Part print with two shaded views. Sizes in mm from the minimum x, y, z corner. Round coordinates to 2 decimals unless told otherwise and drop trailing zeros. Write each loop counter-clockwise with the first axis right and the second up, starting at its lowest first coordinate (ties: lowest second). Pieces come first, ordered by that corner, then holes. Notation, with made-up numbers: M 72,71.25 L 87,71.25 A21 ccw 87,105.25 Z; hole C 33.5,-6 d5. An arc over 180 degrees is marked long. One line per question, with ' | ' between items. Start each with the question number.
1) Saw through at C-C (z = 8.75). List the corners of the cut face in (x, y), plus the area to 3 significant figures.
2) Wall check: probe 1 along X at (y, z) = (135, 9.5); probe 2 along X at (y, z) = (136.5, 7.75); probe 3 along Y at (x, z) = (4.25, 7.25). Give the ranges that are in metal, low to high. Write a range as [from, to].
3) Saw through at B-B (y = 135). List the corners of the cut face in (x, z), plus the area to 4 significant figures.
4) Drop a flat-ended pin along its axis: pin 1 Ø4 at (x, y) = (5.5, 106) entering from -Z. Give the stop position or say it passes through.
5) Mould opens along Y. For the marked faces 1, 2 and 3 say: pulls with the +Y half, pulls with the -Y half, needs draft (parallel to the pull), parting line crosses it, or undercut.
6) Saw through at A-A (x = 15). List the corners of the cut face in (y, z).
7) Saw through at D-D (y = 28.5). List the corners of the cut face in (x, z).
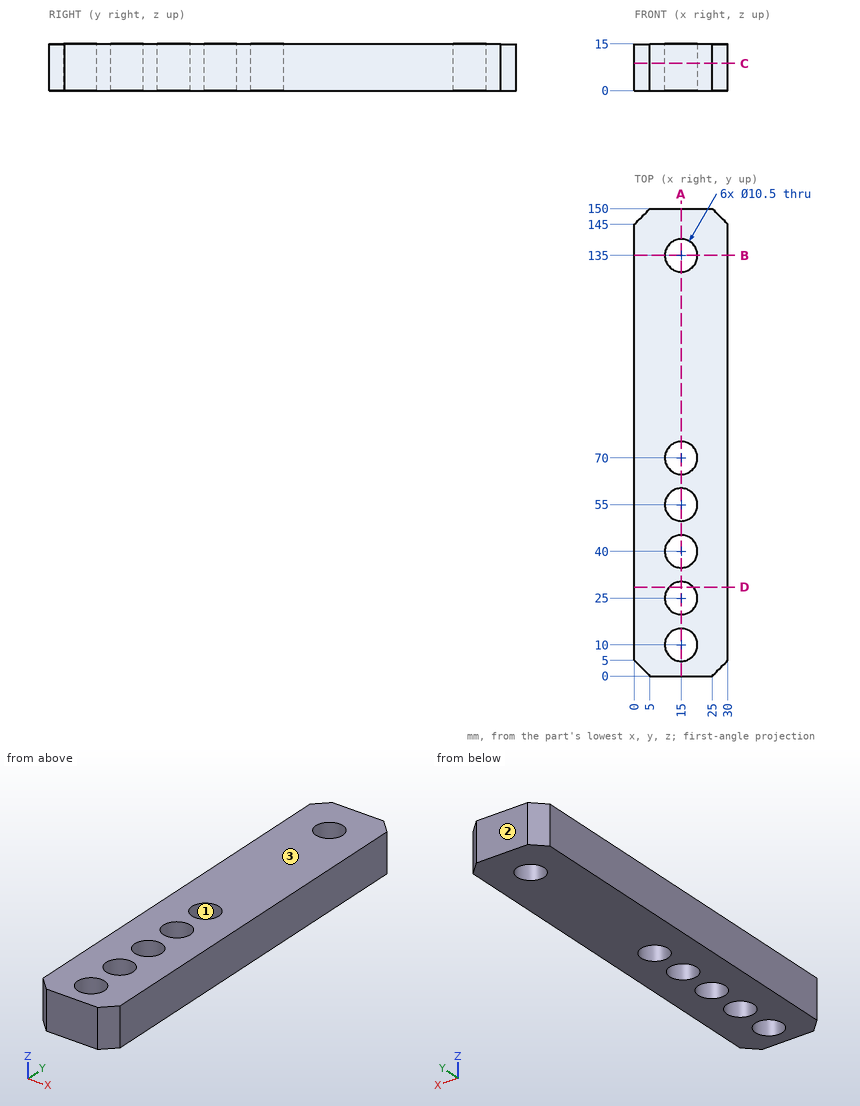
Answer key:
1) outline: M 0,5 L 5,0 L 25,0 L 30,5 L 30,145 L 25,150 L 5,150 L 0,145 Z; hole C 15,10 d10.5; hole C 15,25 d10.5; hole C 15,40 d10.5; hole C 15,55 d10.5; hole C 15,70 d10.5; hole C 15,135 d10.5 | area: 3,930 mm2
2) probe 1: x = [0, 9.75], [20.25, 30] | probe 2: x = [0, 9.97], [20.03, 30] | probe 3: y = [0.75, 149.25]
3) outline: M 0,0 L 9.75,0 L 9.75,15 L 0,15 Z; M 20.25,0 L 30,0 L 30,15 L 20.25,15 Z | area: 292.5 mm2
4) pin 1: stops at z = 0
5) face 1: undercut | face 2: pulls with the +Y half | face 3: needs draft
6) outline: M 0,0 L 4.75,0 L 4.75,15 L 0,15 Z; M 15.25,0 L 19.75,0 L 19.75,15 L 15.25,15 Z; M 30.25,0 L 34.75,0 L 34.75,15 L 30.25,15 Z; M 45.25,0 L 49.75,0 L 49.75,15 L 45.25,15 Z; M 60.25,0 L 64.75,0 L 64.75,15 L 60.25,15 Z; M 75.25,0 L 129.75,0 L 129.75,15 L 75.25,15 Z; M 140.25,0 L 150,0 L 150,15 L 140.25,15 Z
7) outline: M 0,0 L 11.09,0 L 11.09,15 L 0,15 Z; M 18.91,0 L 30,0 L 30,15 L 18.91,15 Z
